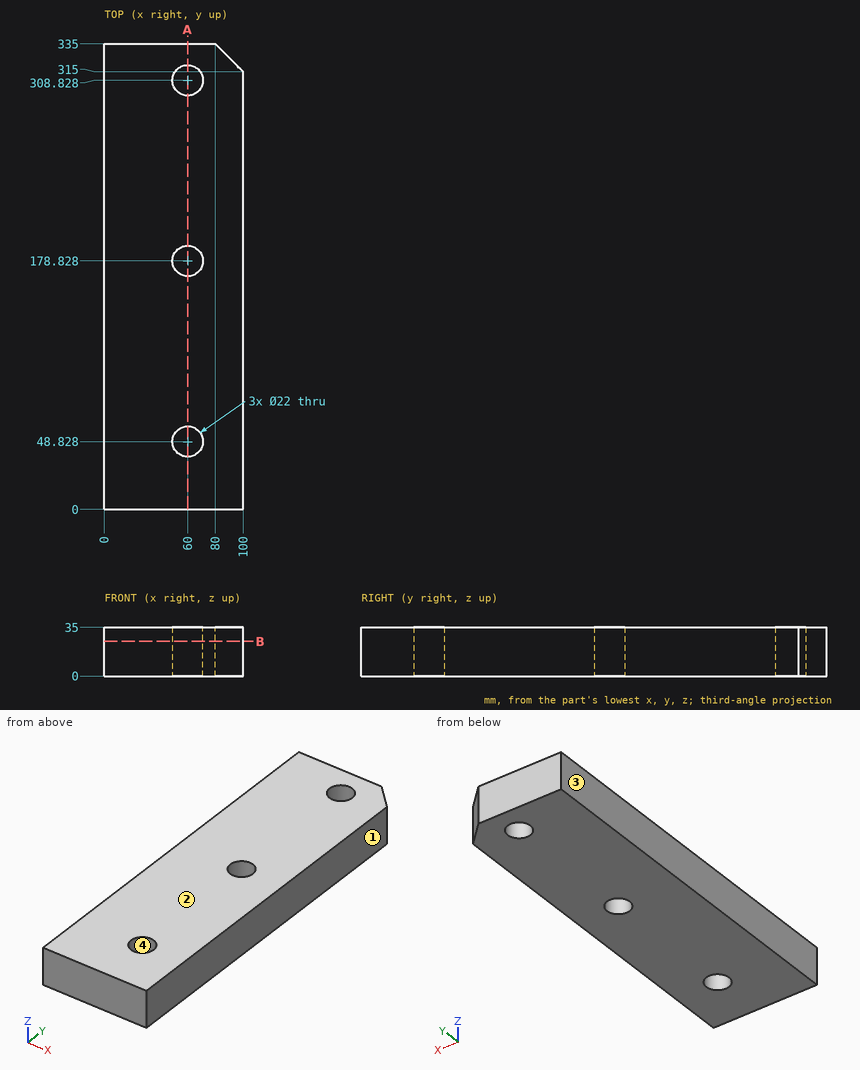
Could you check a few things on this drawing? It's one solid part, dimensions in mm from its lowest x, y, z. Round coordinates to 2 decimals unless told otherwise and drop trailing zeros. Loops run counter-clockwise (first coordinate to the right, second up) from the corner with the lowest first, then second, coordinate; pieces in that order, holes last. Notation, with made-up numbers: (-15, 59.25) -> (2, 59.25) arc R27 ccw to (2, 93.25) -> close; hole circle Ø9 at (13.25, 25). An arc over 180 degrees is marked (long way). Write each question's results on one line, items separated by ' | '.
(1) If we section it at B-B, the plane z = 25: List the corners of the cut face in (x, y) for me.
Worked answers:
outline: (0, 0) -> (100, 0) -> (100, 315) -> (80, 335) -> (0, 335) -> close; hole circle Ø22 at (60, 48.83); hole circle Ø22 at (60, 178.83); hole circle Ø22 at (60, 308.83)
(2) If I drill on L1, parallel to Y at x = 61, z = 28.5; L2, parallel to Y at x = 60, z = 16; L3, parallel to X at y = 51, z = 11.5, over which ranges is the centre line in solid material (lowest first)?
Worked answers:
L1: 0 to 37.87, 59.78 to 167.87, 189.78 to 297.87, 319.78 to 335 | L2: 0 to 37.83, 59.83 to 167.83, 189.83 to 297.83, 319.83 to 335 | L3: 0 to 49.22, 70.78 to 100
(3) If we section it at A-A, the plane x = 60: List the corners of the cut face in (y, z) for me.
Worked answers:
outline: (0, 0) -> (37.83, 0) -> (37.83, 35) -> (0, 35) -> close; (59.83, 0) -> (167.83, 0) -> (167.83, 35) -> (59.83, 35) -> close; (189.83, 0) -> (297.83, 0) -> (297.83, 35) -> (189.83, 35) -> close; (319.83, 0) -> (335, 0) -> (335, 35) -> (319.83, 35) -> close
(4) We'd pull the mould along X, two halves only. Please class the marked faces 1, 2, 3 and 4: released by +X, released by -X, zero draft, split by the parting line, or undercut.
Worked answers:
face 1: released by +X | face 2: zero draft | face 3: released by -X | face 4: undercut
